CAD build for the part. Positions are in the model's coordinates, mm. Face numbers are marked on the shaded views. Round coordinates to 2 decimals unless told otherwise and drop trailing zeros. Order: outer loops, then holes, each group sorted by start corner. A loop starts at its lowest first (then second) coordinate and runs counter-clockwise, first axis right, second up. Notation, with made-up numbers: M 37.25,71.25 L 64.25,71.25 A17 cw 64.25,91.25 Z; hole C 46,43 d3. An arc over 180 degrees is marked long. Put each result on its own line as item: value.
```python
from build123d import *

# Parameters (mm, degrees)
BOSS_EXTRUDE1_DEPTH = 26
SKETCH2_R           = 32.5
CUT_EXTRUDE1_DEPTH  = 2.5
CUT_EXTRUDE2_START  = -2.5
SKETCH3_R           = 32.5
CUT_EXTRUDE2_DEPTH  = 2.5
CHAMFER1_SIZE       = 0.3
HOLE1_D             = 9
HOLE2_D             = 4
HOLE2_DEPTH         = 34
HOLE4_D             = 8
HOLE4_DEPTH         = 6
CUT_EXTRUDE4_DEPTH  = 6


with BuildPart() as part:
    # Sketch1 → Boss-Extrude1 (new body)
    with BuildSketch(Plane.XY):
        with BuildLine():
            Line((-50, 0), (-30, 0))
            ThreePointArc((-30, 0), (0, -30), (30, 0))
            Line((30, 0), (50, 0))
            Line((50, 0), (50, -43))
            Line((50, -43), (-50, -43))
            Line((-50, -43), (-50, 0))
        make_face()
    extrude(amount=BOSS_EXTRUDE1_DEPTH)

    # Sketch2 → Cut-Extrude1 (cut)
    with BuildSketch(Plane.XY.offset(26)):
        Circle(SKETCH2_R)
    extrude(amount=-CUT_EXTRUDE1_DEPTH, mode=Mode.SUBTRACT)

    # Sketch3 → Cut-Extrude2 (cut)
    with BuildSketch(Plane(origin=(0, 0, 0), x_dir=(-1, 0, 0), z_dir=(0, 0, -1)).offset(CUT_EXTRUDE2_START)):
        Circle(SKETCH3_R)
    extrude(amount=CUT_EXTRUDE2_DEPTH, mode=Mode.SUBTRACT)

    # Chamfer1
    chamfer1_edges = [part.edges().sort_by_distance(p)[0] for p in [
        (0, -30, 23.5),
        (0, -30, 2.5),
    ]]
    chamfer(chamfer1_edges, length=CHAMFER1_SIZE)

    # Hole1 (through all)
    with Locations(Plane(origin=(0, 0, 0), x_dir=(1, 0, 0), z_dir=(0, 1, 0))):
        with Locations((-41, -13), (41, -13)):
            Hole(HOLE1_D / 2)

    # Hole2
    with Locations(Plane(origin=(0, 0, 0), x_dir=(1, 0, 0), z_dir=(0, 1, 0))):
        with Locations((0, -13)):
            Hole(HOLE2_D / 2, depth=HOLE2_DEPTH)

    # Hole4
    with Locations(Plane(origin=(0, -43, 0), x_dir=(-1, 0, 0), z_dir=(0, -1, 0))):
        with Locations((-21, -13)):
            Hole(HOLE4_D / 2, depth=HOLE4_DEPTH)

    # Sketch11 → Cut-Extrude4 (cut)
    with BuildSketch(Plane.XZ.offset(43)):
        with BuildLine():
            Line((-20, 17), (-22, 17))
            ThreePointArc((-22, 17), (-26, 13), (-22, 9))
            Line((-22, 9), (-20, 9))
            ThreePointArc((-20, 9), (-16, 13), (-20, 17))
        make_face()
    extrude(amount=-CUT_EXTRUDE4_DEPTH, mode=Mode.SUBTRACT)


solid = part.part
```
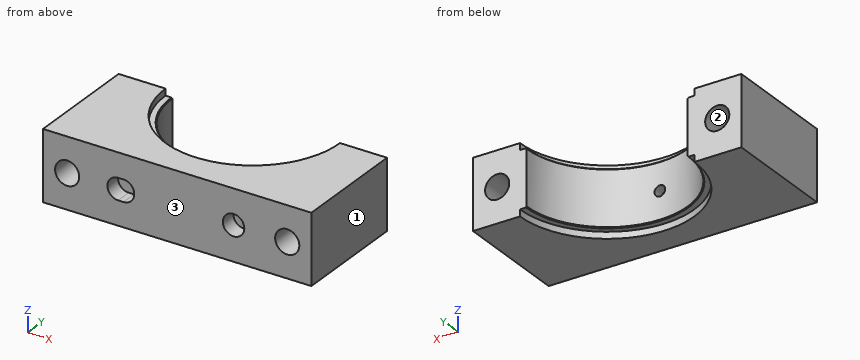
Item 1: Band-saw the part on B-B on z = 13. Give the cut face in (x, y), and give its area (3 significant figures).
Answers below:
outline: M -50,-43 L -45.5,-43 L -45.5,0 L -50,0 Z; M -36.5,-43 L -26,-43 L -26,-37 L -16,-37 L -16,-43 L 17,-43 L 17,-37 L 25,-37 L 25,-43 L 36.5,-43 L 36.5,0 L 30,0 A30 cw 2,-29.93 L 2,-34 L -2,-34 L -2,-29.93 A30 cw -30,0 L -36.5,0 Z; M 45.5,-43 L 50,-43 L 50,0 L 45.5,0 Z
area: 1,990 mm²
Item 2: Band-saw the part on C-C on y = -35. Give the cut face in (x, z), and give its area (3 significant figures).
Answers below:
outline: M -50,0 L 50,0 L 50,26 L -50,26 Z; hole C -41,13 d9; hole C 41,13 d9
area: 2,470 mm²
Item 3: Probe line 1 along Z through (x, y) = (21, -38); line 2 along Z through (x, y) = (0, -32.05); line 3 along X through (y, z) = (-14, 9.5). List the from-to ranges inside material, lowest first. Write a range as [from, to].
Answers below:
line 1: [0, 9], [17, 26]
line 2: [2.5, 11], [15, 23.5]
line 3: [-50, -43.83], [-38.17, -26.53], [26.53, 38.17], [43.83, 50]
Item 4: Band-saw the part on A-A on x = -41. Give the cut face in (y, z).
Answers below:
outline: M -43,0 L 0,0 L 0,8.5 L -43,8.5 Z; M -43,17.5 L 0,17.5 L 0,26 L -43,26 Z
Item 5: Mould opens along X. For the marked faces 1, 2 and 3 say: pulls with the +X half, pulls with the -X half, needs draft (parallel to the pull), parting line crosses it, or undercut.
Answers below:
face 1: pulls with the +X half
face 2: undercut
face 3: needs draft
Item 6: Band-saw the part on D-D on y = -13.5. State how many separate pieces and enclosed holes the cut face has, and give its area (3 significant figures).
Answers below:
separate pieces: 2
enclosed holes: 2
area: 1,050 mm²
Item 7: Pin check, flat tips, straight feed: P1, Ø5, axis at x = 23, z = 12, coming from the +Y side; P2, Ø16.5, axis at x = -3.5, y = -21.5, coming from the +Z side; P3, Ø2.5, axis at x = 21.5, z = 14.5, coming from the -Y side; P4, Ø5.5, axis at x = 41, z = 13, coming from the +Y side. Stop position of each tip, or through.
Answers below:
P1: y = -15.8
P2: z = 23.23
P3: y = -37
P4: through
